The listing builds one solid part. Answer for the finished solid, in the listing's coordinates (mm). A direction names the side the tool comes from. Coordinates: 2 decimals unless noted, no trailing zeros. Write each loop counter-clockwise with the first axis right and the second up, starting at its lowest first coordinate (ties: lowest second). Pieces come first, ordered by that corner, then holes. Notation, with made-up numbers: M 43,63.25 L 50,63.25 A29 ccw 50,100.25 Z; hole C -0.75,2 d4. An arc over 180 degrees is marked long. Write item = value, one per line. Start each with the question number.
```python
from build123d import *

# Parameters (mm, degrees)
RING_PROFILE_23_20_R      = 11.5
RING_PROFILE_23_20_R_2    = 10
RING_23X12_DEPTH          = 6
STEM_PROFILE_R            = 6
STEM_DEPTH                = 18
RING_START                = -18
RING_CUT_PROFILE_R        = 10
RING_CUT_DEPTH            = 18
SIDE_BOSS_PROFILE_9_R     = 4.5
SIDE_BOSS_9_DEPTH         = 6
SIDE_HOLE_PROFILE_3_R     = 1.5
SIDE_HOLE_3_DEPTH         = 6
COUNTERBORE_PROFILE_6_R   = 3
COUNTERBORE_PROFILE_6_R_2 = 1.5
COUNTERBORE_6X2_DEPTH     = 2
STEM_TRIM_CUT_DEPTH       = 12


with BuildPart() as part:
    # Ring Profile Ø23-Ø20 → Ring Ø23x12 (new, symmetric)
    with BuildSketch(Plane.XY):
        Circle(RING_PROFILE_23_20_R)
        Circle(RING_PROFILE_23_20_R_2, mode=Mode.SUBTRACT)
    extrude(amount=RING_23X12_DEPTH, both=True)

    # Stem Profile → Stem (add)
    with BuildSketch(Plane(origin=(0, -25, 0), x_dir=(-1, 0, 0), z_dir=(0, -1, 0))):
        with Locations(Location((0, 0, 0), (0, 0, 180))):
            Circle(STEM_PROFILE_R)
        with BuildLine():
            Line((-1.5, -3.708099244), (1.5, -3.708099244))
            ThreePointArc((1.5, -3.708099244), (0, 4), (-1.5, -3.708099244))
        make_face(mode=Mode.SUBTRACT)
    extrude(amount=-STEM_DEPTH)

    # Ring Cut Profile → Ring Cut (cut)
    with BuildSketch(Plane.XY.offset(6).offset(RING_START)):
        Circle(RING_CUT_PROFILE_R)
    extrude(amount=RING_CUT_DEPTH, mode=Mode.SUBTRACT)

    # Side Boss Profile Ø9 → Side Boss Ø9 (add)
    with BuildSketch(Plane.XY.offset(8)):
        with Locations((0, -19)):
            Circle(SIDE_BOSS_PROFILE_9_R)
    extrude(amount=-SIDE_BOSS_9_DEPTH)

    # Side Hole Profile Ø3 → Side Hole Ø3 (cut)
    with BuildSketch(Plane.XY.offset(8)):
        with Locations((0, -19)):
            Circle(SIDE_HOLE_PROFILE_3_R)
    extrude(amount=-SIDE_HOLE_3_DEPTH, mode=Mode.SUBTRACT)

    # Counterbore Profile Ø6 → Counterbore Ø6x2 (cut)
    with BuildSketch(Plane.XY.offset(8)):
        with Locations((0, -19)):
            Circle(COUNTERBORE_PROFILE_6_R)
        with Locations((0, -19)):
            Circle(COUNTERBORE_PROFILE_6_R_2, mode=Mode.SUBTRACT)
    extrude(amount=-COUNTERBORE_6X2_DEPTH, mode=Mode.SUBTRACT)

    # Stem Trim Profile → Stem Trim Cut (cut)
    with BuildSketch(Plane.XZ.offset(25)):
        with BuildLine():
            Line((-1.5, 3.708099244), (1.5, 3.708099244))
            ThreePointArc((1.5, 3.708099244), (0, -4), (-1.5, 3.708099244))
        make_face()
    extrude(amount=-STEM_TRIM_CUT_DEPTH, mode=Mode.SUBTRACT)


solid = part.part
```
1. The part is cut by section C-C, the plane z = 4.5. Write down the section's boundary in (x, y).
2. For a pull along X with two mould halves and no side action, classify faces 1 (the face through (-2.17, -9.76, -0.08)), 2 (the face through (-9, 5, 6)), 3 (the face through (-1.5, 11.4, 0.1)) as pulls with the +X half, pulls with the -X half, needs draft (parallel to the pull), parting line crosses it, or undercut.
3. The part is cut by section B-B, the plane x = 8. Write down the section's boundary in (y, z), and give its area (3 significant figures).
4. The part is cut by section D-D, the plane y = -21. Write down the section's boundary in (x, z), and give its area (3 significant figures).
5. Straight lines are drawn through the part: L1, parallel to X at y = -22, z = -0.25; L2, parallel to Y at x = 0, z = 6.8; L3, parallel to X at y = 0, z = 1. For each, find the intervals that lie inside material, in ascending order. Write a range as [from, to].
6. The part is cut by section A-A, the plane y = 0. Write down the section's boundary in (x, z).
7. Each of these flat-tipped pins is pushed along its axis until it touches: pin 1 (3.5 mm diameter, centred on x = 0, y = -19, fed in from +Z); pin 2 (1.5 mm diameter, centred on x = -6, y = -19, fed in from -Z); pin 3 (1 mm diameter, centred on y = -9, z = 1, fed in from +X). Where does it stop, or does it pass through?
8. For faces 4 (the face through (-9, 5, -6)), 5 (the face through (1, -22, 8)), 6 (the face through (-1.301, -17.512, -5.857)), 7 (the face through (-0.59, -14.54, 6.46)), 8 (the face through (0, -23, 3.708)), determine the directions among +Z, -Z, +X, -X, +Y, -Y from which every point of the face is accessible in a straight line to the end or side of a thin tool.
Solution:
q1.outline = M -3.97,-25 L 3.97,-25 L 3.97,-21.12 A4.5 ccw 3.97,-16.88 L 3.97,-10.79 A11.5 ccw long -3.97,-10.79 L -3.97,-16.88 A4.5 ccw -3.97,-21.12 Z; hole C 0,0 d20; hole C 0,-19 d3
q2.face_1 = undercut
q2.face_2 = needs draft
q2.face_3 = parting line crosses it
q3.outline = M -8.26,-6 L -6,-6 L -6,6 L -8.26,6 Z; M 6,-6 L 8.26,-6 L 8.26,6 L 6,6 Z
q3.area = 54.3 mm^2
q4.outline = M -4.03,4.44 A6 ccw long 4.03,4.44 L 4.03,8 L 2.24,8 L 2.24,6 L -2.24,6 L -2.24,8 L -4.03,8 Z; hole M -1.5,3.71 A4 ccw long 1.5,3.71 Z
q4.area = 74.5 mm^2
q5.L1 = [-5.99, -3.99], [3.99, 5.99]
q5.L2 = [-23.5, -22], [-16, -14.5]
q5.L3 = [-11.5, -10], [10, 11.5]
q6.outline = M -11.5,-6 L -10,-6 L -10,6 L -11.5,6 Z; M 10,-6 L 11.5,-6 L 11.5,6 L 10,6 Z
q7.pin_1 = 6
q7.pin_2 = -2.9
q7.pin_3 = 7.75
q8.face_4 = -Z, +X, -X, +Y, -Y
q8.face_5 = +Z, +X, -X, +Y, -Y
q8.face_6 = none
q8.face_7 = +Z
q8.face_8 = -Y
